Read the model definition and answer for the solid it produces. Units are mm, in the model's axes. A direction names the side the tool comes from. Coordinates: 2 decimals unless noted, no trailing zeros. Order: outer loops, then holes, each group sorted by start corner. A loop starts at its lowest first (then second) coordinate and runs counter-clockwise, first axis right, second up. Notation, with made-up numbers: M 36.25,-32 L 75.25,-32 A29 cw 75.25,-6 Z; hole C -40,-4 d4. An arc over 180 degrees is marked long. Use a Markdown table: item, result. Add a question column.
1) The mould has two halves that part along Z. Classify faces 4 (the face through (47, -22, 5)), 5 (the face through (25, -6, 0)), 6 (the face through (41, -6.5, 5)), 7 (the face through (10.2, -3.2, 3.5)): released by +Z, released by -Z, zero draft, split by the parting line, or undercut.
2) Find section B-B on x = 39. Write down the section's boundary in (y, z), plus the area to 3 significant figures.
3) Find section D-D on y = -17.75. Write down the section's boundary in (x, z), plus the area to 3 significant figures.
4) Find the intervals of material crossed by probe 1 along X at (y, z) = (-17.5, 1); probe 2 along Z at (x, y) = (39, -8.95); probe 3 along Y at (x, z) = (16, 2.5), in increasing order. Write a range as [from, to].
5) Find section A-A on y = -4. Write down the section's boundary in (x, z).
6) Each of these flat-tipped pins is pushed along its axis until it touches: pin 1 Ø5 at (x, z) = (39, 5) entering from -Y; pin 2 Ø5 at (x, z) = (37.5, 4) entering from -Y; pin 3 Ø3 at (x, z) = (11, 5) entering from +Y. Where does it stop, or does it pass through?
7) For faces 1 (the face through (25, -6, 10)), 2 (the face through (5, -17, 5)), 3 (the face through (8.6, -8.3, 3.2)), determine the directions among +Z, -Z, +X, -X, +Y, -Y from which every point of the face is accessible in a straight line to the end or side of a thin tool.
8) Find section C-C on z = 5. Count the separate pieces of the cut face and the enclosed holes in it, plus the area to 3 significant figures.
from build123d import *

# Parameters (mm, degrees)
BOSS_EXTRUDE1_DEPTH                     = 10
CBORE_FOR_M3_HEX_HEAD_BOLT1_D           = 3.4
CBORE_FOR_M3_HEX_HEAD_BOLT1_CBORE_D     = 6
CBORE_FOR_M3_HEX_HEAD_BOLT1_CBORE_DEPTH = 3.5
FILLET1_R                               = 2
FILLET2_R                               = 0.5
CHAMFER1_SIZE                           = 2


with BuildPart() as part:
    # Sketch1 → Boss-Extrude1 (new body)
    with BuildSketch(Plane.XY):
        Polygon((45, -22), (50, -22), (50, 0), (0, 0), (0, -22), (5, -22), (5, -10), (45, -10), align=None)
    extrude(amount=BOSS_EXTRUDE1_DEPTH)

    # CBORE for M3 Hex Head Bolt1 (through all)
    with Locations(Plane.XZ.offset(10)):
        with Locations((11, 5), (39, 5)):
            CounterBoreHole(CBORE_FOR_M3_HEX_HEAD_BOLT1_D / 2, CBORE_FOR_M3_HEX_HEAD_BOLT1_CBORE_D / 2, CBORE_FOR_M3_HEX_HEAD_BOLT1_CBORE_DEPTH)

    # Fillet1
    fillet1_edges = [part.edges().sort_by_distance(p)[0] for p in [
        (45, -10, 5),
        (5, -10, 5),
    ]]
    fillet(fillet1_edges, radius=FILLET1_R)

    # Fillet2
    fillet2_edges = [part.edges().sort_by_distance(p)[0] for p in [
        (50, -22, 5),
        (45, -22, 5),
        (5, -22, 5),
        (0, -22, 5),
    ]]
    fillet(fillet2_edges, radius=FILLET2_R)

    # Chamfer1
    chamfer1_edges = [part.edges().sort_by_distance(p)[0] for p in [
        (0, 0, 5),
        (50, 0, 5),
    ]]
    chamfer(chamfer1_edges, length=CHAMFER1_SIZE)


solid = part.part
Check result:
| question | item | result |
|---|---|---|
| 1 | face 4 | zero draft |
| 1 | face 5 | released by -Z |
| 1 | face 6 | undercut |
| 1 | face 7 | undercut |
| 2 | outline | M -10,0 L 0,0 L 0,3.3 L -6.5,3.3 L -6.5,2 L -10,2 Z; M -10,8 L -6.5,8 L -6.5,6.7 L 0,6.7 L 0,10 L -10,10 Z |
| 2 | area | 56.9 mm2 |
| 3 | outline | M 0,0 L 5,0 L 5,10 L 0,10 Z; M 45,0 L 50,0 L 50,10 L 45,10 Z |
| 3 | area | 100 mm2 |
| 4 | probe 1 | x = [0, 5], [45, 50] |
| 4 | probe 2 | z = [0, 2], [8, 10] |
| 4 | probe 3 | y = [-10, 0] |
| 5 | outline | M 0,0 L 50,0 L 50,10 L 0,10 Z; hole C 11,5 d3.4; hole C 39,5 d3.4 |
| 6 | pin 1 | stops at y = -6.5 |
| 6 | pin 2 | stops at y = -10 |
| 6 | pin 3 | passes through |
| 7 | face 1 | +Z, +X, -X, +Y, -Y |
| 7 | face 2 | +Z, -Z, -Y |
| 7 | face 3 | -Y |
| 8 | separate pieces | 3 |
| 8 | enclosed holes | 0 |
| 8 | area | 531 mm2 |
